```python
from build123d import *

# Parameters (mm, degrees)
CIRPATTERN1_COUNT  = 4
CHAMFER1_SIZE      = 0.4
CUT_EXTRUDE1_START = -10
SKETCH6_R          = 32.5
SKETCH6_R_2        = 32.25
CUT_EXTRUDE1_DEPTH = 10


with BuildPart() as part:
    # Sketch1 → Revolve1 (revolve)
    with BuildSketch(Plane.XY, mode=Mode.PRIVATE) as revolve1_sk:
        Polygon((0, 16), (1.695369244, 16), (1.695369244, 16.85), (2.995369244, 16.85), (2.995369244, 16), (13, 16), (13, 12.5), (15, 12.5), (15, 0), (18, 0), (18, 32.5), (14, 32.5), (14, 20), (0, 20), align=None)
    revolve(revolve1_sk.sketch.rotate(Axis((15, 0, 0), (1, 0, 0)), 90), axis=Axis((15, 0, 0), (1, 0, 0)))

    # Sketch2 → Cut-Revolve1 (revolve, cut)
    with BuildSketch(Plane(origin=(0, 0, 0), x_dir=(1, 0, 0), z_dir=(0, 1, 0)), mode=Mode.PRIVATE) as cut_revolve1_sk:
        Polygon((14, 26.5), (18, 26.5), (18, 31), (15.75, 28.75), (14, 28.75), align=None)
    cut_revolve1 = revolve(cut_revolve1_sk.sketch.rotate(Axis((14, 0, -26.5), (1, 0, 0)), 180), axis=Axis((14, 0, -26.5), (1, 0, 0)), mode=Mode.SUBTRACT)

    # CirPattern1: Cut-Revolve1 ×4 about axis
    cirpattern1_axis = Axis((0, 0, 0), (1, 0, 0))
    for i in range(1, CIRPATTERN1_COUNT):
        add(cut_revolve1.rotate(cirpattern1_axis, i * 360 / CIRPATTERN1_COUNT), mode=Mode.SUBTRACT)

    # Chamfer1
    chamfer1_edges = [part.edges().sort_by_distance(p)[0] for p in [
        (14, 0, -32.5),
        (18, 0, -32.5),
        (13, 0, -12.5),
        (0, 0, -16),
        (0, 0, -20),
    ]]
    chamfer(chamfer1_edges, length=CHAMFER1_SIZE)

    # Sketch6 → Cut-Extrude1 (cut)
    with BuildSketch(Plane(origin=(18, 0, 0), x_dir=(0, 0, -1), z_dir=(1, 0, 0)).offset(CUT_EXTRUDE1_START)):
        Circle(SKETCH6_R)
        Circle(SKETCH6_R_2, mode=Mode.SUBTRACT)
    extrude(amount=CUT_EXTRUDE1_DEPTH, mode=Mode.SUBTRACT)


solid = part.part
```
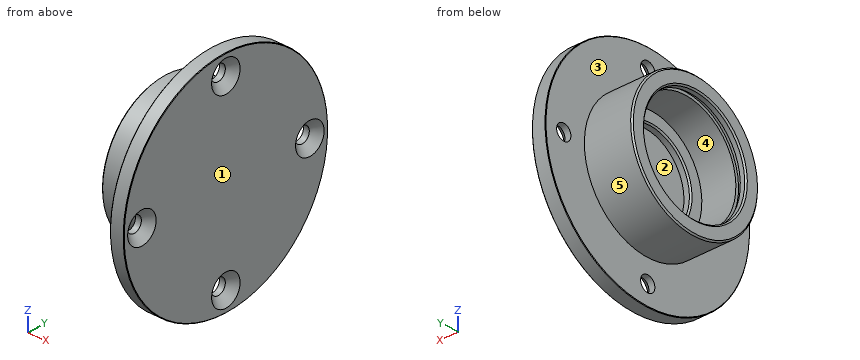
Design review of the part built by this model. Coordinates are the model's own, in mm. Face numbers are marked on the shaded views. A direction names the side the tool comes from. Coordinates: 2 decimals unless noted, no trailing zeros. Write each loop counter-clockwise with the first axis right and the second up, starting at its lowest first coordinate (ties: lowest second). Pieces come first, ordered by that corner, then holes.
1) Add section A-A (x = 8.5). Write out the cut boundary in (y, z), plus the area to 3 significant figures.
2) Insertion check: pin 1 (7.5 mm diameter, centred on y = -1.5, z = -5.5, fed in from -X); pin 2 (6 mm diameter, centred on y = 0, z = -26.5, fed in from -X); pin 3 (5 mm diameter, centred on x = 9.5, y = -1, fed in from +Z). Each pin has a flat end and moves straight along its axis. Give the tip position at first contact, or say it passes through.
3) Machinability: for the marked faces 1 and 2, which of the approach directions +Z, -Z, +X, -X, +Y, -Y give a long, thin tool a straight path to every point of the face, cutting with its end or side? Answer none if there is none.
4) Add section C-C (x = 17). Write out the cut boundary in (y, z), plus the area to 3 significant figures.
5) Mouldability with a two-part tool opening along Y and no side actions: class the marked faces 3, 4 and 5 as +Y half, -Y half, draft (parallel to the pull), parting line (faces both ways), or undercut.
6) To check wall thickness, follow L1, parallel to Y at x = 2.45, z = 0; L2, parallel to Y at x = 8.25, z = 0; L3, parallel to X at y = -6, z = -12.5. State the ranges of each line that lie inside material, in increasing order.
7) Add section B-B (z = 0). State how many separate pieces and enclosed holes the cut face has, plus the area to 3 significant figures.
Check result:
1. outline: circle Ø40 at (0, 0); hole circle Ø32 at (0, 0)
1. area: 452 mm2
2. pin 1: stops at x = 15
2. pin 2: stops at x = 14
2. pin 3: stops at z = 20
3. face 1: +Z, -Z, +X, +Y, -Y
3. face 2: -X
4. outline: circle Ø64.5 at (0, 0); hole circle Ø7 at (-26.5, 0); hole circle Ø7 at (0, -26.5); hole circle Ø7 at (0, 26.5); hole circle Ø7 at (26.5, 0)
4. area: 3,110 mm2
5. face 3: draft
5. face 4: undercut
5. face 5: parting line
6. L1: y = -20 to -16.85, 16.85 to 20
6. L2: y = -20 to -16, 16 to 20
6. L3: x = 13 to 18
7. separate pieces: 3
7. enclosed holes: 0
7. area: 303 mm2
